from build123d import *

# Parameters (mm, degrees)
EXTRUDE_1_DEPTH      = 12.5
EXTRUDE_1_DEPTH_BACK = 12.5
SKETCH_1_W           = 25
SKETCH_1_H           = 25
EXTRUDE_2_DEPTH      = 24.5
EXTRUDE_2_DEPTH_BACK = 24.5
SKETCH_4_R           = 5
EXTRUDE_3_DEPTH      = 24.5
EXTRUDE_3_DEPTH_BACK = 24.5
SKETCH_5_R           = 5


with BuildPart() as part:
    # 草图1 → 凸台-拉伸1 (new, two sides: drawn at the far end of the back side and taken through both)
    with BuildSketch(Plane(origin=(0, 0, 0), x_dir=(0, 0, -1), z_dir=(1, 0, 0)).offset(-EXTRUDE_1_DEPTH_BACK)):
        Rectangle(SKETCH_1_W, SKETCH_1_H)
    extrude(amount=EXTRUDE_1_DEPTH + EXTRUDE_1_DEPTH_BACK)

    # 草图2 → 切除-旋转1 (revolve, cut)
    with BuildSketch(Plane(origin=(0, 0, 0), x_dir=(0, 0, -1), z_dir=(1, 0, 0))):
        with BuildLine():
            Line((0, -25), (-25, -25))
            Line((-25, -25), (-25, 9.090909091))
            ThreePointArc((-25, 9.090909091), (-17.67766953, -8.586760439), (0, -15.909090909))
            Line((0, -15.909090909), (0, -25))
        make_face()
    revolve(axis=Axis((0, -15.909090909, 0), (0, -1, 0)), mode=Mode.SUBTRACT)

    # 草图3 → 切除-旋转2 (revolve, cut)
    with BuildSketch(Plane(origin=(0, 0, 0), x_dir=(0, 0, -1), z_dir=(1, 0, 0))):
        with BuildLine():
            Line((0, 25), (25, 25))
            Line((25, 25), (25, -9.090909091))
            ThreePointArc((25, -9.090909091), (17.67766953, 8.586760439), (0, 15.909090909))
            Line((0, 15.909090909), (0, 25))
        make_face()
    revolve(axis=Axis((0, 15.909090909, 0), (0, 1, 0)), mode=Mode.SUBTRACT)

    # 草图4 → 凸台-拉伸2 (add, two sides: drawn at the far end of the back side and taken through both)
    with BuildSketch(Plane(origin=(0, 0, 0), x_dir=(1, 0, 0), z_dir=(0, 1, 0)).offset(-EXTRUDE_2_DEPTH_BACK)):
        with Locations(Location((0, 0, 0), (0, 0, 270))):
            Circle(SKETCH_4_R)
    extrude(amount=EXTRUDE_2_DEPTH + EXTRUDE_2_DEPTH_BACK)

    # 草图5 → 凸台-拉伸3 (add, two sides: drawn at the far end of the back side and taken through both)
    with BuildSketch(Plane(origin=(0, 0, 0), x_dir=(0, 0, -1), z_dir=(1, 0, 0)).offset(-EXTRUDE_3_DEPTH_BACK)):
        Circle(SKETCH_5_R)
    extrude(amount=EXTRUDE_3_DEPTH + EXTRUDE_3_DEPTH_BACK)


solid = part.part
Design review of the part built by this model. Coordinates are the model's own, in mm. A direction names the side the tool comes from. Give positions to 0.01 mm unless a question says otherwise; leave off trailing zeros. Write each loop counter-clockwise with the first axis right and the second up, starting at its lowest first coordinate (ties: lowest second). Pieces come first, ordered by that corner, then holes. Notation, with made-up numbers: M 46,37 L 55,37 A28 cw 55,67 Z; hole C 83.5,6.25 d4. An arc over 180 degrees is marked long. Answer as a JSON object with one key per item and string values. Group by question number.
1) For line 1 along X through (y, z) = (13, 0.25); line 2 along Y through (x, z) = (3, 9), list the stretches that pass through material, from the lowest coordinate up.
2) Tool access review of faces 1 (the face through (-18.58, -4.88, 1.08)), 2 (the face through (12.5, -5.4, 0.2)), 3 (the face through (5.4, -12.5, 0.2)): name each direction out of +Z, -Z, +X, -X, +Y, -Y from which nothing blocks a thin tool from reaching the whole face with its end or side.
3) We need section B-B (z = 0). Give the boundary of the cut face in (x, y), and give its area (4 significant figures).
4) Clearance check with flat-ended pins moving along their axes: pin 1 Ø6 at (y, z) = (-10, 6) entering from +X; pin 2 Ø12 at (x, z) = (16.5, -5.5) entering from +Y; pin 3 Ø1.5 at (y, z) = (14.5, 5) entering from +X; pin 4 Ø4 at (y, z) = (-16.5, -8.5) entering from +X. State where each tip first meets the part, or that it passes through.
5) We need section D-D (y = -18.5). Give the boundary of the cut face in (x, z).
6) We need section A-A (y = 0). Give the boundary of the cut face in (x, z).
Answer key:
{
 "1": {"line 1": "x = -4.99 to 4.99", "line 2": "y = -12.5 to 12.5"},
 "2": {"face 1": "-X", "face 2": "+X", "face 3": "-Y"},
 "3": {"outline": "M -24.5,-5 L -12.5,-5 L -12.5,-12.5 L -5,-12.5 L -5,-24.5 L 5,-24.5 L 5,-12.5 L 12.5,-12.5 L 12.5,-5 L 24.5,-5 L 24.5,5 L 12.5,5 L 12.5,12.5 L 5,12.5 L 5,24.5 L -5,24.5 L -5,12.5 L -12.5,12.5 L -12.5,5 L -24.5,5 Z", "area": "1,105 mm²"},
 "4": {"pin 1": "stops at x = 12.5", "pin 2": "stops at y = 12.5", "pin 3": "stops at x = 2.63", "pin 4": "passes through"},
 "5": {"outline": "C 0,0 d10"},
 "6": {"outline": "M -24.5,-5 L -12.5,-5 L -12.5,-12.5 L 12.5,-12.5 L 12.5,-5 L 24.5,-5 L 24.5,5 L 12.5,5 L 12.5,12.5 L -12.5,12.5 L -12.5,5 L -24.5,5 Z"}
}
